CAD build for the part. Positions are in the model's coordinates, mm. A direction names the side the tool comes from. Coordinates: 2 decimals unless noted, no trailing zeros. Write each loop counter-clockwise with the first axis right and the second up, starting at its lowest first coordinate (ties: lowest second). Pieces come first, ordered by that corner, then holes. Notation, with made-up numbers: M -19.75,50 L 32.25,50 A28 cw 32.25,70 Z; hole C 44,23 d6. An arc over 180 degrees is marked long. Put each result on its own line as item: value. Start each with the question number.
```python
from build123d import *

# Parameters (mm, degrees)
SKETCH1_R            = 3.95
BOSS_EXTRUDE1_DEPTH  = 8
SKETCH2_W            = 2
SKETCH2_H            = 1.5
BOSS_EXTRUDE2_DEPTH  = 3
FILLET1_R            = 0.2
SKETCH3_R            = 3.9
BOSS_EXTRUDE3_DEPTH  = 0.2
SKETCH4_R            = 4.5
BOSS_EXTRUDE4_DEPTH  = 7.6
SKETCH6_R            = 3.9
BOSS_EXTRUDE5_DEPTH  = 0.2
CHAMFER2_SIZE        = 0.2
SKETCH7_R            = 4
BOSS_EXTRUDE8_DEPTH  = 10
SKETCH9_R            = 3.5
BOSS_EXTRUDE9_DEPTH  = 20
SKETCH10_R           = 3
BOSS_EXTRUDE10_DEPTH = 10
SKETCH13_R           = 2.75
BOSS_EXTRUDE11_DEPTH = 15
BOSS_EXTRUDE13_DEPTH = 3
FILLET2_R            = 0.2
CHAMFER5_SIZE        = 0.1


with BuildPart() as part:
    # Sketch1 → Boss-Extrude1 (new body)
    with BuildSketch(Plane.XY):
        Circle(SKETCH1_R)
    extrude(amount=BOSS_EXTRUDE1_DEPTH)

    # Sketch2 → Boss-Extrude2 (add)
    with BuildSketch(Plane(origin=(0, 0, 5), x_dir=(-1, 0, 0), z_dir=(0, 0, -1))):
        with Locations((0, 3.75)):
            Rectangle(SKETCH2_W, SKETCH2_H)
    extrude(amount=-BOSS_EXTRUDE2_DEPTH)

    # Fillet1
    fillet1_edges = [part.edges().sort_by_distance(p)[0] for p in [
        (-1, 4.5, 6.5),
        (1, 4.5, 6.5),
    ]]
    fillet(fillet1_edges, radius=FILLET1_R)

    # Sketch3 → Boss-Extrude3 (add)
    with BuildSketch(Plane(origin=(0, 0, 0), x_dir=(-1, 0, 0), z_dir=(0, 0, -1))):
        Circle(SKETCH3_R)
    extrude(amount=BOSS_EXTRUDE3_DEPTH)

    # Sketch4 → Boss-Extrude4 (add)
    with BuildSketch(Plane(origin=(0, 0, -0.2), x_dir=(-1, 0, 0), z_dir=(0, 0, -1))):
        with Locations(Location((0, 0, 0), (0, 0, 180))):
            Circle(SKETCH4_R)
    extrude(amount=BOSS_EXTRUDE4_DEPTH)

    # Sketch6 → Boss-Extrude5 (add)
    with BuildSketch(Plane(origin=(0, 0, -7.8), x_dir=(-1, 0, 0), z_dir=(0, 0, -1))):
        Circle(SKETCH6_R)
    extrude(amount=BOSS_EXTRUDE5_DEPTH)

    # Chamfer2
    chamfer2_edges = [part.edges().sort_by_distance(p)[0] for p in [
        (-2.413762623, -3.126699538, 8),
    ]]
    chamfer(chamfer2_edges, length=CHAMFER2_SIZE)

    # Sketch7 → Boss-Extrude8 (add)
    with BuildSketch(Plane(origin=(0, 0, -8), x_dir=(-1, 0, 0), z_dir=(0, 0, -1))):
        Circle(SKETCH7_R)
    extrude(amount=BOSS_EXTRUDE8_DEPTH)

    # Sketch9 → Boss-Extrude9 (add)
    with BuildSketch(Plane(origin=(0, 0, -18), x_dir=(-1, 0, 0), z_dir=(0, 0, -1))):
        Circle(SKETCH9_R)
    extrude(amount=BOSS_EXTRUDE9_DEPTH)

    # Sketch10 → Boss-Extrude10 (add)
    with BuildSketch(Plane(origin=(0, 0, -38), x_dir=(-1, 0, 0), z_dir=(0, 0, -1))):
        Circle(SKETCH10_R)
    extrude(amount=BOSS_EXTRUDE10_DEPTH)

    # Sketch13 → Boss-Extrude11 (add)
    with BuildSketch(Plane(origin=(0, 0, -48), x_dir=(-1, 0, 0), z_dir=(0, 0, -1))):
        Circle(SKETCH13_R)
    extrude(amount=BOSS_EXTRUDE11_DEPTH)

    # Sketch14 → Boss-Extrude13 (add)
    with BuildSketch(Plane(origin=(0, 0, -60), x_dir=(-1, 0, 0), z_dir=(0, 0, -1))):
        with BuildLine():
            Line((-1, 3.5), (1, 3.5))
            Line((1, 3.5), (1, 2.561737691))
            ThreePointArc((1, 2.561737691), (0, 2.75), (-1, 2.561737691))
            Line((-1, 2.561737691), (-1, 3.5))
        make_face()
    extrude(amount=BOSS_EXTRUDE13_DEPTH)

    # Fillet2
    fillet2_edges = [part.edges().sort_by_distance(p)[0] for p in [
        (-1, 3.5, -61.5),
        (1, 3.5, -61.5),
    ]]
    fillet(fillet2_edges, radius=FILLET2_R)

    # Chamfer5
    chamfer5_edges = [part.edges().sort_by_distance(p)[0] for p in [
        (-4.5, 0, -0.2),
        (-4.5, 0, -7.8),
        (4, 0, -18),
        (3.5, 0, -38),
        (3, 0, -48),
        (1.551209206, -2.270737766, -63),
    ]]
    chamfer(chamfer5_edges, length=CHAMFER5_SIZE)


solid = part.part
```
(1) Which spindle directions (+Z, -Z, +X, -X, +Y, -Y) get a long thin tool onto all of the face, cutting with end or side? Do faces 1 (the face through (0, 3.5, -61)), 2 (the face through (0, 0, -63)), 3 (the face through (-3, 3, -7.8)). Say none if no direction does.
(2) Drill centre lines: line 1 (Z direction, x = -2.75, y = 0.75); line 2 (X direction, y = 0.25, z = -19); line 3 (Y direction, x = -0.75, z = -51.5). Where is each one in solid material? Low to high. Write a range as [from, to].
(3) Slice it at B-B, the plane z = -23. Write the cut outline in (x, y).
(4) Slice it at A-A, the plane z = -10.5. Write the cut outline in (x, y).
(5) Drop flat-ended pins along their axis: pin 1 (3 mm diameter, centred on x = -0.5, z = -23, fed in from -Y); pin 2 (3 mm diameter, centred on x = -3, y = -3.5, fed in from +Z); pin 3 (5 mm diameter, centred on y = -1, z = -47.5, fed in from -X); pin 4 (4 mm diameter, centred on x = -0.5, z = -48, fed in from +Y). Give the stop position or say it passes through.
Result set:
1. face 1: -Z, +X, -X, +Y
1. face 2: -Z, +X, -X, +Y, -Y
1. face 3: none
2. line 1: z = [-48, 8]
2. line 2: x = [-3.49, 3.49]
2. line 3: y = [-2.65, 2.65]
3. outline: C 0,0 d7
4. outline: C 0,0 d8
5. pin 1: stops at y = -3.5
5. pin 2: stops at z = 8
5. pin 3: stops at x = -3
5. pin 4: stops at y = 3
